The listing builds one solid part. Answer for the finished solid, in the listing's coordinates (mm). Face numbers are marked on the shaded views. Coordinates: 2 decimals unless noted, no trailing zeros. Loops run counter-clockwise (first coordinate to the right, second up) from the corner with the lowest first, then second, coordinate; pieces in that order, holes last. Notation, with made-up numbers: (65, 53) -> (103, 53) arc R30 ccw to (103, 78) -> close; hole circle Ø10 at (-16, 10). An arc over 180 degrees is marked (long way). Answer in a Markdown table with one row per item.
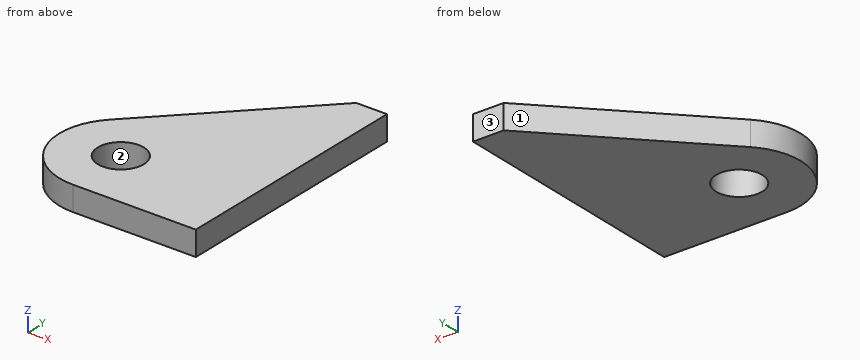
```python
from build123d import *

# Parameters (mm, degrees)
SKETCH1_R           = 7.5
BOSS_EXTRUDE1_DEPTH = 4


with BuildPart() as part:
    # Sketch1 → Boss-Extrude1 (new, symmetric)
    with BuildSketch(Plane.XY):
        with BuildLine():
            Line((0, 0), (0, 80))
            Line((0, 80), (-10, 80))
            Line((-10, 80), (-54.4083313, 33.870832317))
            ThreePointArc((-54.4083313, 33.870832317), (-58.404030079, 12.171099896), (-40, 0))
            Line((-40, 0), (0, 0))
        make_face()
        with Locations((-40, 20)):
            Circle(SKETCH1_R, mode=Mode.SUBTRACT)
    extrude(amount=BOSS_EXTRUDE1_DEPTH, both=True)


solid = part.part
```
Item 1: Find the intervals of material crossed by probe 1 along X at (y, z) = (24, 1); probe 2 along X at (y, z) = (14.5, 2.75); probe 3 along Y at (x, z) = (-44.5, 2.5), in increasing order.
Findings below:
| item | result |
|---|---|
| probe 1 | x = -59.6 to -46.34, -33.66 to 0 |
| probe 2 | x = -59.23 to -45.1, -34.9 to 0 |
| probe 3 | y = 0.51 to 14, 26 to 44.16 |
Item 2: A cutting plane is placed at C-C, the plane x = -49.5. Determine the outline of the cut face in (y, z).
Findings below:
| item | result |
|---|---|
| outline | (2.4, -4) -> (38.97, -4) -> (38.97, 4) -> (2.4, 4) -> close |
Item 3: Determine the mould class of the marked faces 1, 2 and 3 for opening direction X: +X half, -X half, draft (parallel to the pull), parting line (faces both ways), or undercut.
Findings below:
| item | result |
|---|---|
| face 1 | -X half |
| face 2 | undercut |
| face 3 | draft |
Item 4: Flat-ended cylindrical pins translate along their axes: pin 1 Ø2 at (x, z) = (-42.5, 1) entering from +Y; pin 2 Ø1 at (x, z) = (-52.5, 3) entering from +Y; pin 3 Ø1 at (y, z) = (23, 2) entering from -X. Find the tip coordinate at first contact, or state that the pin passes through.
Findings below:
| item | result |
|---|---|
| pin 1 | stops at y = 47.28 |
| pin 2 | stops at y = 36.37 |
| pin 3 | stops at x = -59.84 |
Item 5: A cutting plane is placed at A-A, the plane y = 20. Determine the outline of the cut face in (x, z), plus the area to 3 significant figures.
Findings below:
| item | result |
|---|---|
| outline | (-60, -4) -> (-47.5, -4) -> (-47.5, 4) -> (-60, 4) -> close; (-32.5, -4) -> (0, -4) -> (0, 4) -> (-32.5, 4) -> close |
| area | 360 mm2 |
Item 6: A cutting plane is placed at B-B, the plane z = -1.75. Determine the outline of the cut face in (x, y).
Findings below:
| item | result |
|---|---|
| outline | (-54.41, 33.87) arc R20 ccw to (-40, 0) -> (0, 0) -> (0, 80) -> (-10, 80) -> close; hole circle Ø15 at (-40, 20) |
Item 7: A cutting plane is placed at D-D, the plane y = 43. Determine the outline of the cut face in (x, z).
Findings below:
| item | result |
|---|---|
| outline | (-45.62, -4) -> (0, -4) -> (0, 4) -> (-45.62, 4) -> close |
